Input: part model. Units: mm. Frame: model coordinates. A direction names the side the tool comes from. Coordinates: 2 decimals unless noted, no trailing zeros. Loops run counter-clockwise (first coordinate to the right, second up) from the corner with the lowest first, then second, coordinate; pieces in that order, holes last.
Item 1: Section B-B on x = 10. Return loops of the section in (y, z), and give its area (3 significant figures).
Item 2: Contact query for flat-ended pins moving along their axis: P1, Ø3, axis at x = 14, z = 2, coming from the -Y side; P2, Ø2, axis at x = 28, y = 4, coming from the -Z side; P3, Ø1, axis at x = 8, y = -6, coming from the +Z side; P4, Ø1, axis at x = 17, z = -4, coming from the +Y side. Output: stop coordinate, or through.
Item 3: Section A-A on x = 4.5. Return loops of the section in (y, z), and give its area (3 significant figures).
Item 4: Ray query, line 1 along X through (y, z) = (-2.75, -6); line 2 along Z through (x, y) = (17.5, -3); line 3 along Z through (x, y) = (12.5, -4.5). Return the intervals inside material, ascending.
Item 5: Reachability of faces 1 (the flat face through (2.859, -6.896, -4.056)), 2 (the flat face through (6.4, -5, -3)) from +Z, -Z, +X, -X, +Y, -Y: full face, straight path, thin tool, end or side. Return the list, or none.
```python
from build123d import *

# Parameters (mm, degrees)
EXTRUDE_387_DEPTH = 6.4
FILLET_1280_R     = 0.4


with BuildPart() as part:
    # 草图1 → Extrude 387 (new body)
    with BuildSketch(Plane(origin=(0, 0, 0), x_dir=(0, 0, -1), z_dir=(1, 0, 0))):
        Polygon((8, 4.618802154), (8, -4.618802154), (0, -9.237604307), (-8, -4.618802154), (-8, 4.618802154), (0, 9.237604307), align=None)
    extrude(amount=EXTRUDE_387_DEPTH)

    # 草图2 → 凸台-旋转1 (revolve)
    with BuildSketch(Plane.XY, mode=Mode.PRIVATE) as revolve_1_sk:
        Polygon((0, 0), (31.4, 0), (31.4, 3.701), (31.4, 5), (16.4, 5), (0, 5), align=None)
    revolve(revolve_1_sk.sketch.rotate(Axis((0, 0, 0), (1, 0, 0)), 90), axis=Axis((0, 0, 0), (1, 0, 0)))

    # 草图3 → 切除-旋转1 (revolve, cut)
    with BuildSketch(Plane.XY):
        Polygon((0, 8), (3.601282526, 14.237604307), (3.601282526, 19.237604307), (-10, 19.237604307), (-10, 8), align=None)
    revolve(axis=Axis((0, 0, 0), (1, 0, 0)), mode=Mode.SUBTRACT)

    # 草图4 → 切除-旋转3 (revolve, cut)
    with BuildSketch(Plane.XY, mode=Mode.PRIVATE) as cut_revolve_3_sk:
        Polygon((6.4, 7.315), (5.8, 7.661410162), (5.8, 9.237604307), (6.4, 9.237604307), align=None)
    revolve(cut_revolve_3_sk.sketch.rotate(Axis((0, 0, 0), (1, 0, 0)), 90), axis=Axis((0, 0, 0), (1, 0, 0)), mode=Mode.SUBTRACT)

    # Fillet 1280
    fillet_1280_edges = [part.edges().sort_by_distance(p)[0] for p in [
        (6.4, 0, -5),
    ]]
    fillet(fillet_1280_edges, radius=FILLET_1280_R)


solid = part.part
```
Results found:
1. outline: circle Ø10 at (0, 0)
1. area: 78.5 mm2
2. P1: stops at y = -4.97
2. P2: stops at z = -4
2. P3: passes through
2. P4: stops at y = 3.57
3. outline: (-9.24, 0) - (-4.62, -8) - (4.62, -8) - (9.24, 0) - (4.62, 8) - (-4.62, 8) - close
3. area: 222 mm2
4. line 1: x = 0 to 6.4
4. line 2: z = -4 to 4
4. line 3: z = -2.18 to 2.18
5. face 1: -Z, +X, -X, -Y
5. face 2: +X
